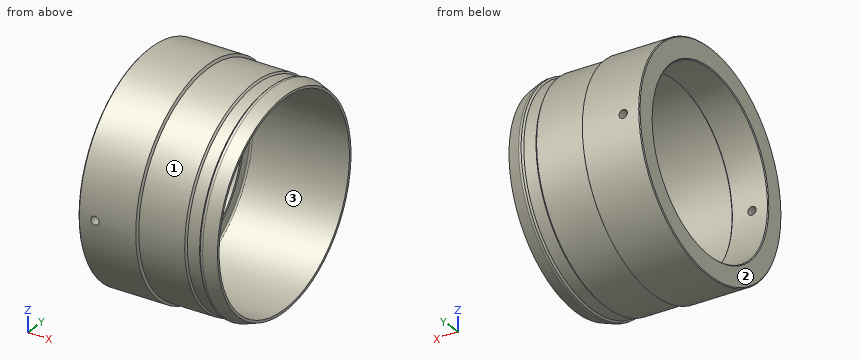
```python
from build123d import *

# Parameters (mm, degrees)
FILLET1_R          = 2
CHAMFER1_SIZE      = 1
M12_TAPPED_HOLE1_D = 10.2


with BuildPart() as part:
    # Sketch1 → Revolve1 (revolve)
    with BuildSketch(Plane.XY, mode=Mode.PRIVATE) as revolve1_sk:
        Polygon((0, 110), (45, 110), (45, 124), (165, 124), (165, 127), (150, 132), (147, 132), (145, 130), (130, 130), (128, 132), (71.732050808, 132), (70, 135), (0, 135), align=None)
    revolve(revolve1_sk.sketch.rotate(Axis((0, 0, 0), (1, 0, 0)), 90), axis=Axis((0, 0, 0), (1, 0, 0)))

    # Fillet1
    fillet1_edges = [part.edges().sort_by_distance(p)[0] for p in [
        (45, 0, -124),
    ]]
    fillet(fillet1_edges, radius=FILLET1_R)

    # Chamfer1
    chamfer1_edges = [part.edges().sort_by_distance(p)[0] for p in [
        (45, 0, -110),
        (0, 0, -110),
        (0, 0, -135),
    ]]
    chamfer(chamfer1_edges, length=CHAMFER1_SIZE)

    # M12 Tapped Hole1 (through all)
    with Locations(Plane(origin=(20, 135, 0), x_dir=(0, 0, 1), z_dir=(0, 1, 0))):
        with Locations((0, 0)):
            Hole(M12_TAPPED_HOLE1_D / 2)


solid = part.part
```
Work out the finished part from the listing and answer in its coordinate system (mm). Face numbers are marked on the shaded views. Give positions to 0.01 mm unless a question says otherwise; leave off trailing zeros. Order: outer loops, then holes, each group sorted by start corner. A loop starts at its lowest first (then second) coordinate and runs counter-clockwise, first axis right, second up. Notation, with made-up numbers: (35.5, 8) - (51.5, 8) arc R16 cw to (51.5, 23) - close; hole circle Ø11 at (-2, 65). An arc over 180 degrees is marked (long way). One line per item, written item: value. Start each with the question number.
1. For a pull along Y with two mould halves and no side action, classify the marked faces 1, 2 and 3 as released by +Y, released by -Y, zero draft, split by the parting line, or undercut.
2. Each of these flat-tipped pins is pushed along its axis until it touches: pin 1 Ø12 at (x, y) = (92.5, 99) entering from +Z (3 decimals); pin 2 Ø3 at (x, z) = (128, 56.5) entering from +Y; pin 3 Ø8 at (x, y) = (138, -16.5) entering from +Z; pin 4 Ø1.5 at (y, z) = (-43, -105.5) entering from -X. Where does it stop, or does it pass through?
3. Consider line 1 (Y direction, x = 32, z = 0); line 2 (Y direction, x = 77, z = 0); line 3 (X direction, y = -120.5, z = 0). Determine where each line is inside the solid, lowest interval first.
4. Section D-D, the plane x = 141.5 is taken. Write down the section's boundary in (y, z).
5. Section C-C, the plane z = 0 is taken. Count the separate pieces of the cut face and the enclosed holes in it, then the cut area to 3 significant figures.
6. Section B-B, the plane x = 20 is taken. Write down the section's boundary in (y, z), then the cut area to 3 significant figures.
Filled sheet:
1. face 1: split by the parting line
1. face 2: zero draft
1. face 3: undercut
2. pin 1: z = 93.675
2. pin 2: y = 120
2. pin 3: z = 129.4
2. pin 4: x = 0
3. line 1: -135 to -110, 110 to 135
3. line 2: -132 to -124, 124 to 132
3. line 3: 0 to 14.9, 25.1 to 45
4. outline: circle Ø260 at (0, 0); hole circle Ø248 at (0, 0)
5. separate pieces: 4
5. enclosed holes: 0
5. area: 3,670 mm²
6. outline: (-134.9, -5.1) arc R135 ccw to (134.9, -5.1) - (109.88, -5.1) arc R110 cw to (-109.88, -5.1) - close; (-134.9, 5.1) - (-109.88, 5.1) arc R110 cw to (109.88, 5.1) - (134.9, 5.1) arc R135 ccw to start
6. area: 18,700 mm²
